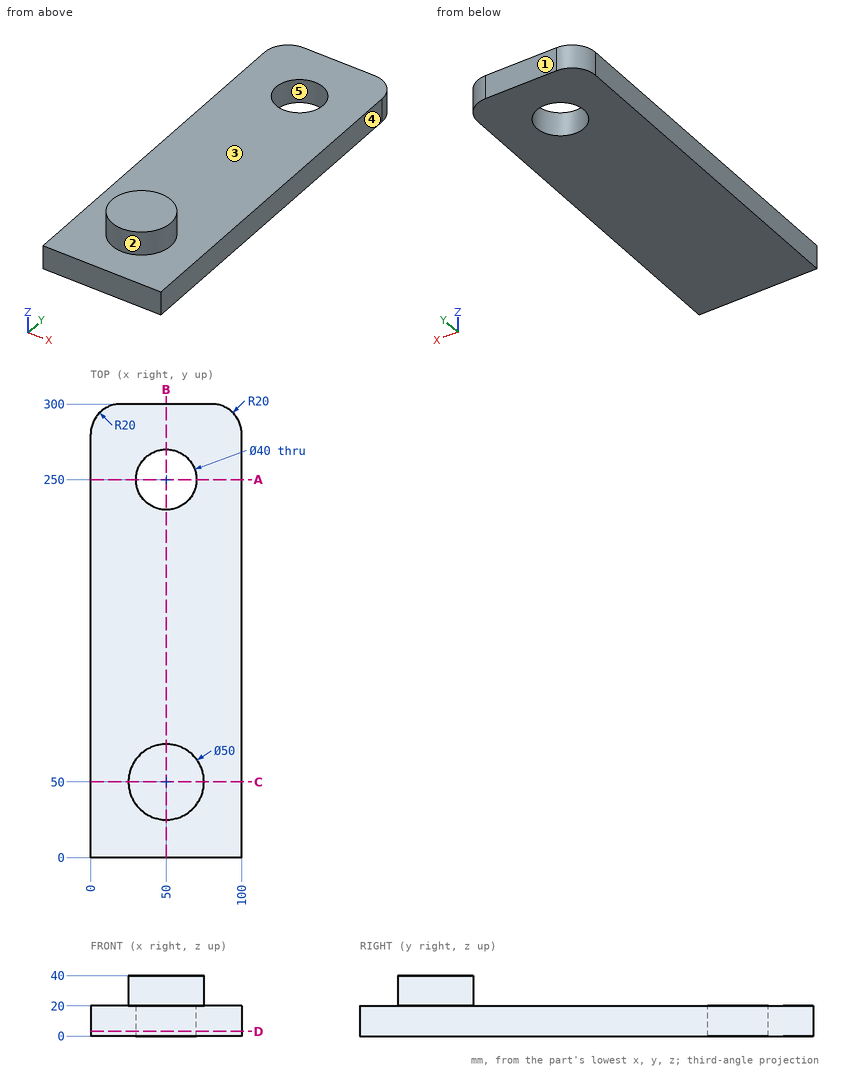
Job drawing, mm, ordinate dimensions from the low corner. One solid piece. A direction names the side the tool comes from. Round coordinates to 2 decimals unless told otherwise and drop trailing zeros. Write each loop counter-clockwise with the first axis right and the second up, starting at its lowest first coordinate (ties: lowest second). Pieces come first, ordered by that corner, then holes.
1) Drill centre lines: probe 1 along Y at (x, z) = (50, 12); probe 2 along Z at (x, y) = (21, 161.5); probe 3 along X at (y, z) = (263, 13.5). Where is each one in solid material? Low to high.
2) Band-saw the part on A-A, the plane y = 250. List the corners of the cut face in (x, z).
3) Band-saw the part on C-C, the plane y = 50. List the corners of the cut face in (x, z).
4) Band-saw the part on D-D, the plane z = 3. List the corners of the cut face in (x, y), and give its area (3 significant figures).
5) Band-saw the part on B-B, the plane x = 50. List the corners of the cut face in (y, z).
6) Pin check, flat tips, straight feed: pin 1 (4 mm diameter, centred on x = 84.5, z = 23, fed in from +Y); pin 2 (1.5 mm diameter, centred on x = 62.5, y = 145.5, fed in from +Z). Stop position of each tip, or through.
7) 3-axis set-ups, long thin cutter, end or side, ignore diameter. For the marked faces 1 and 2: which of +Z, -Z, +X, -X, +Y, -Y reach the whole face in a straight line?
8) Mould opens along X. For the marked faces 3, 4 and 5 say: +X half, -X half, draft (parallel to the pull), parting line (faces both ways), or undercut.
Ans:
1. probe 1: y = 0 to 230, 270 to 300
1. probe 2: z = 0 to 20
1. probe 3: x = 0 to 34.8, 65.2 to 100
2. outline: (0, 0) - (30, 0) - (30, 20) - (0, 20) - close; (70, 0) - (100, 0) - (100, 20) - (70, 20) - close
3. outline: (0, 0) - (100, 0) - (100, 20) - (75, 20) - (75, 40) - (25, 40) - (25, 20) - (0, 20) - close
4. outline: (0, 0) - (100, 0) - (100, 280) arc R20 ccw to (80, 300) - (20, 300) arc R20 ccw to (0, 280) - close; hole circle Ø40 at (50, 250)
4. area: 28,600 mm2
5. outline: (0, 0) - (230, 0) - (230, 20) - (75, 20) - (75, 40) - (25, 40) - (25, 20) - (0, 20) - close; (270, 0) - (300, 0) - (300, 20) - (270, 20) - close
6. pin 1: passes through
6. pin 2: stops at z = 20
7. face 1: +Z, -Z, +X, -X, +Y
7. face 2: +Z
8. face 3: draft
8. face 4: +X half
8. face 5: undercut
